```python
from build123d import *

# Parameters (mm, degrees)
BOSS_EXTRUDE1_DEPTH = 3


with BuildPart() as part:
    # Sketch1 → Boss-Extrude1 (new body)
    with BuildSketch(Plane.XY):
        with BuildLine():
            Line((-360, -3), (-385, -3))
            Line((-385, -3), (-385, 27))
            Line((-385, 27), (-405, 27))
            ThreePointArc((-405, 27), (-408.535533906, 25.535533906), (-410, 22))
            Line((-410, 22), (-410, -3))
            Line((-410, -3), (-410, -23))
            ThreePointArc((-410, -23), (-408.535533906, -26.535533906), (-405, -28))
            Line((-405, -28), (-365, -28))
            ThreePointArc((-365, -28), (-361.464466094, -26.535533906), (-360, -23))
            Line((-360, -23), (-360, -3))
        make_face()
    extrude(amount=BOSS_EXTRUDE1_DEPTH)


solid = part.part
```
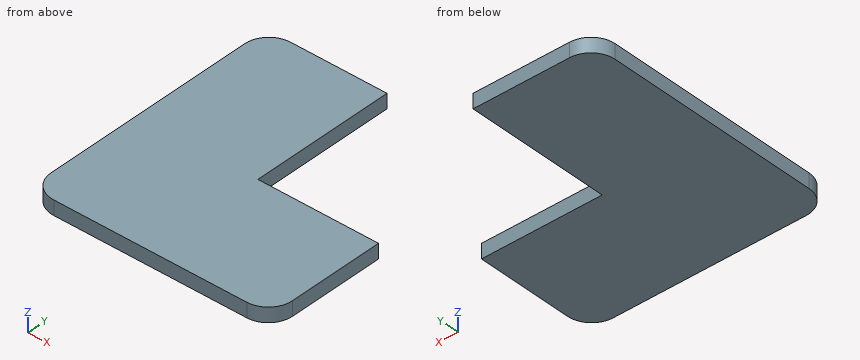
Can you work these out from the model? Positions are in its coordinate system, mm. Coordinates: 2 decimals unless noted, no trailing zeros. Order: outer loops, then holes, each group sorted by start corner. A loop starts at its lowest first (then second) coordinate and runs counter-clockwise, first axis right, second up.
1. If we section it at A-A (z = 2.35): Please give me the cut outline in (x, y), then the cut area to 3 significant figures.
2. If we section it at C-C (x = -381.5): Please give me the cut outline in (y, z), then the cut area to 3 significant figures.
3. I need wall thicknesses on line 1 (X direction, y = 20, z = 1.95); line 2 (Y direction, x = -381, z = 2.3); line 3 (X direction, y = -23.5, z = 1.55). Which ranges of each line are inside material? Lowest first, please.
4. If we section it at B-B (y = 20.5): Please give me the cut outline in (x, z).
5. I'm going to push flat-ended pins straight in: pin 1 (5 mm diameter, centred on x = -389, y = 2, fed in from -Z); pin 2 (0.9 mm diameter, centred on x = -372.5, z = 1.5, fed in from +Y). Where does each tip first touch, or does it pass through?
Entries:
1. outline: (-410, -23) arc R5 ccw to (-405, -28) - (-365, -28) arc R5 ccw to (-360, -23) - (-360, -3) - (-385, -3) - (-385, 27) - (-405, 27) arc R5 ccw to (-410, 22) - close
1. area: 1,980 mm2
2. outline: (-28, 0) - (-3, 0) - (-3, 3) - (-28, 3) - close
2. area: 75.0 mm2
3. line 1: x = -410 to -385
3. line 2: y = -28 to -3
3. line 3: x = -409.97 to -360.03
4. outline: (-410, 0) - (-385, 0) - (-385, 3) - (-410, 3) - close
5. pin 1: stops at z = 0
5. pin 2: stops at y = -3
